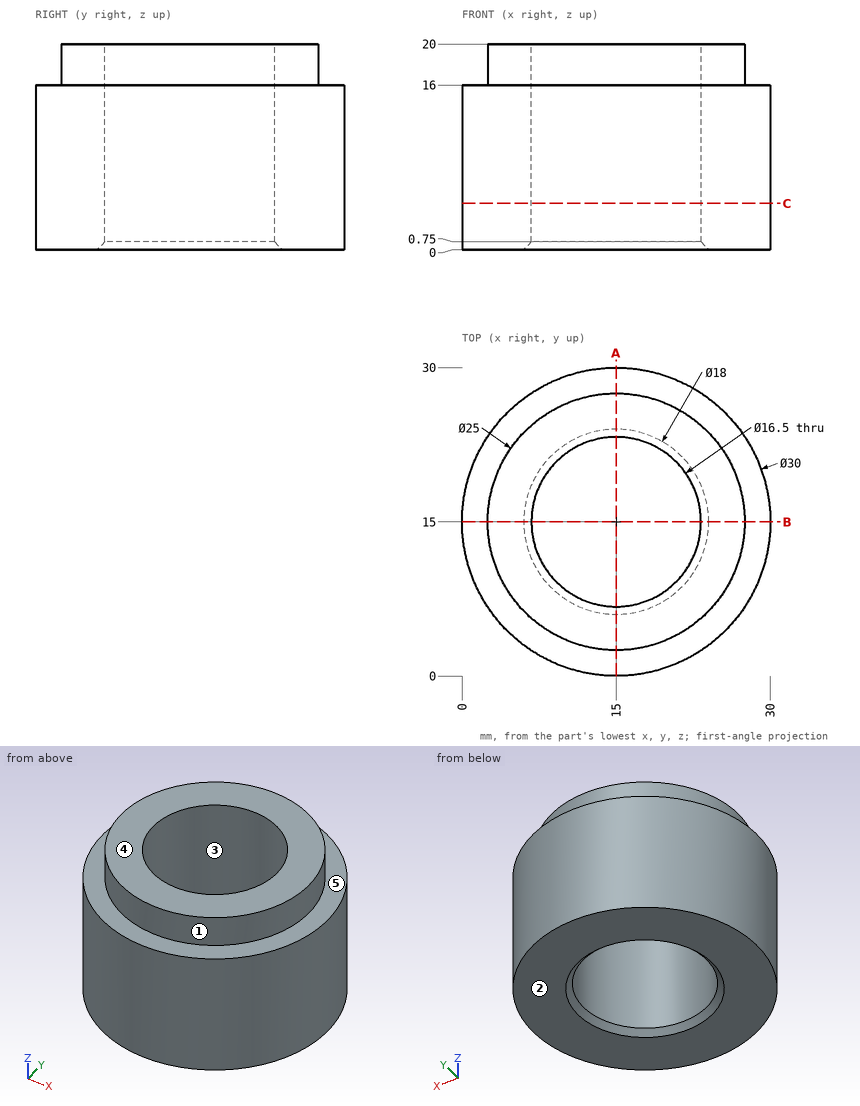
Source: three-view drawing plus pictorial views. Frame: mm from the lowest corner of the part. A direction names the side the tool comes from. Round coordinates to 2 decimals unless told otherwise and drop trailing zeros. Order: outer loops, then holes, each group sorted by start corner. A loop starts at its lowest first (then second) coordinate and runs counter-clockwise, first axis right, second up. Notation, with made-up numbers: (45, -35) - (74, -35) arc R19 cw to (74, -25) - close; hole circle Ø2 at (15, 56.5). An arc over 180 degrees is marked (long way). Answer in a Markdown table with one row per item.
Item 1: Line query: line 1 (Y direction, x = 15, z = 5.5); line 2 (Z direction, x = 15, y = 29.25); line 3 (Y direction, x = 8, z = 5.25). Output: solid intervals per line, ascending.
Model answer:
| item | result |
|---|---|
| line 1 | y = 0 to 6.75, 23.25 to 30 |
| line 2 | z = 0 to 16 |
| line 3 | y = 1.73 to 10.63, 19.37 to 28.27 |
Item 2: Section query C-C (z = 4.5). Return the cut outline in (x, y).
Model answer:
| item | result |
|---|---|
| outline | circle Ø30 at (15, 15); hole circle Ø16.5 at (15, 15) |
Item 3: Reachability of the marked faces 4 and 5 from +Z, -Z, +X, -X, +Y, -Y: full face, straight path, thin tool, end or side. Return the list, or none.
Model answer:
| item | result |
|---|---|
| face 4 | +Z, +X, -X, +Y, -Y |
| face 5 | +Z |
Item 4: Mould query, pull axis X, two halves, no side actions, for the marked faces 1, 2 and 3. Classes: released by +X, released by -X, zero draft, split by the parting line, or undercut.
Model answer:
| item | result |
|---|---|
| face 1 | split by the parting line |
| face 2 | zero draft |
| face 3 | undercut |
Item 5: Section query A-A (x = 15). Return the cut outline in (y, z).
Model answer:
| item | result |
|---|---|
| outline | (0, 0) - (6, 0) - (6.75, 0.75) - (6.75, 20) - (2.5, 20) - (2.5, 16) - (0, 16) - close; (23.25, 0.75) - (24, 0) - (30, 0) - (30, 16) - (27.5, 16) - (27.5, 20) - (23.25, 20) - close |
Item 6: Pin query (flat end, axial travel): pin 1 (5 mm diameter, centred on y = 10, z = 6, fed in from -X); pin 2 (1 mm diameter, centred on x = 17, z = 15.5, fed in from -Y); pin 3 (2 mm diameter, centred on x = 5, z = 13.5, fed in from +Y). Return the tip coordinate at first contact, or that it passes through.
Model answer:
| item | result |
|---|---|
| pin 1 | stops at x = 0.21 |
| pin 2 | stops at y = 0.08 |
| pin 3 | stops at y = 27 |
